from build123d import *

# Parameters (mm, degrees)
BOSS_EXTRUDE1_DEPTH = 20
SKETCH2_R           = 32.5
CUT_EXTRUDE1_DEPTH  = 2.5
CUT_EXTRUDE2_START  = -2.5
SKETCH3_R           = 32.5
CUT_EXTRUDE2_DEPTH  = 2.5
CHAMFER1_SIZE       = 0.3
HOLE1_D             = 9
HOLE2_D             = 4
HOLE2_DEPTH         = 34


with BuildPart() as part:
    # Sketch1 → Boss-Extrude1 (new body)
    with BuildSketch(Plane.XY):
        with BuildLine():
            Line((-50, 0), (-30, 0))
            ThreePointArc((-30, 0), (0, -30), (30, 0))
            Line((30, 0), (50, 0))
            Line((50, 0), (50, -43))
            Line((50, -43), (-50, -43))
            Line((-50, -43), (-50, 0))
        make_face()
    extrude(amount=BOSS_EXTRUDE1_DEPTH)

    # Sketch2 → Cut-Extrude1 (cut)
    with BuildSketch(Plane.XY.offset(20)):
        Circle(SKETCH2_R)
    extrude(amount=-CUT_EXTRUDE1_DEPTH, mode=Mode.SUBTRACT)

    # Sketch3 → Cut-Extrude2 (cut)
    with BuildSketch(Plane(origin=(0, 0, 0), x_dir=(-1, 0, 0), z_dir=(0, 0, -1)).offset(CUT_EXTRUDE2_START)):
        Circle(SKETCH3_R)
    extrude(amount=CUT_EXTRUDE2_DEPTH, mode=Mode.SUBTRACT)

    # Chamfer1
    chamfer1_edges = [part.edges().sort_by_distance(p)[0] for p in [
        (0, -30, 17.5),
        (0, -30, 2.5),
    ]]
    chamfer(chamfer1_edges, length=CHAMFER1_SIZE)

    # Hole1 (through all)
    with Locations(Plane(origin=(0, 0, 0), x_dir=(1, 0, 0), z_dir=(0, 1, 0))):
        with Locations((-41, -10), (41, -10)):
            Hole(HOLE1_D / 2)

    # Hole2
    with Locations(Plane(origin=(0, 0, 0), x_dir=(1, 0, 0), z_dir=(0, 1, 0))):
        with Locations((0, -10)):
            Hole(HOLE2_D / 2, depth=HOLE2_DEPTH)


solid = part.part
Verification items for the finished model (mm, model axes). A direction names the side the tool comes from. Coordinates: 2 decimals unless noted, no trailing zeros. Loops run counter-clockwise (first coordinate to the right, second up) from the corner with the lowest first, then second, coordinate; pieces in that order, holes last. Notation, with made-up numbers: (58, 68) -> (80, 68) arc R5 ccw to (80, 74) -> close; hole circle Ø1 at (48, 31.25). An arc over 180 degrees is marked (long way). Write each question's results on one line, items separated by ' | '.
Item 1: Tool access check on faces 4 (the face through (0, -31, 17.5)), 5 (the face through (0, -34, 10)), 6 (the face through (0, -31, 2.5)). Record the directions out of +Z, -Z, +X, -X, +Y, -Y that give a thin tool (end or side, any length) a straight path to the whole face; none if there is none.
Found:
face 4: +Z, +Y | face 5: +Y | face 6: -Z, +Y
Item 2: Section check C-C, the plane y = -31.5. Enter the section's corners in (x, z).
Found:
outline: (-50, 0) -> (-8, 0) -> (-8, 2.5) -> (8, 2.5) -> (8, 0) -> (50, 0) -> (50, 20) -> (8, 20) -> (8, 17.5) -> (-8, 17.5) -> (-8, 20) -> (-50, 20) -> close; hole circle Ø9 at (-41, 10); hole circle Ø4 at (0, 10); hole circle Ø9 at (41, 10)
Item 3: Gauge pin test, flat end, axial feed: pin 1 (1.2 mm diameter, centred on x = -1, z = 10, fed in from +Y). Record the tip position at first contact, or that the pin passes through.
Found:
pin 1: stops at y = -34
Item 4: Mould release check, pull along X, two halves, no side actions. Record for faces 1 (the face through (-50, -22, 10)), 2 (the face through (36.708, -21.801, 8.648)), 3 (the face through (1, -43, 10)): +X half, -X half, draft (parallel to the pull), parting line (faces both ways), or undercut.
Found:
face 1: -X half | face 2: undercut | face 3: draft
Item 5: Section check D-D, the plane z = 4.5. Enter the section's corners in (x, y), plus the area to 3 significant figures.
Found:
outline: (-50, -43) -> (50, -43) -> (50, 0) -> (30, 0) arc R30 cw to (-30, 0) -> (-50, 0) -> close | area: 2,890 mm2
Item 6: Section check B-B, the plane x = -41. Enter the section's corners in (y, z), plus the area to 3 significant figures.
Found:
outline: (-43, 0) -> (0, 0) -> (0, 5.5) -> (-43, 5.5) -> close; (-43, 14.5) -> (0, 14.5) -> (0, 20) -> (-43, 20) -> close | area: 473 mm2
Item 7: Material ranges on L1, parallel to Z at x = 0, y = -31.2; L2, parallel to Z at x = -41, y = -25.5; L3, parallel to X at y = -27.5, z = 9.25, recorded low to high.
Found:
L1: z = 2.5 to 8, 12 to 17.5 | L2: z = 0 to 5.5, 14.5 to 20 | L3: x = -50 to -45.44, -36.56 to -11.99, 11.99 to 36.56, 45.44 to 50
Item 8: Section check A-A, the plane z = 10. Enter the section's corners in (x, y), plus the area to 3 significant figures.
Found:
outline: (-50, -43) -> (-45.5, -43) -> (-45.5, 0) -> (-50, 0) -> close; (-36.5, -43) -> (36.5, -43) -> (36.5, 0) -> (30, 0) arc R30 cw to (2, -29.93) -> (2, -34) -> (-2, -34) -> (-2, -29.93) arc R30 cw to (-30, 0) -> (-36.5, 0) -> close; (45.5, -43) -> (50, -43) -> (50, 0) -> (45.5, 0) -> close | area: 2,100 mm2
